Could you check a few things on this model? Use its own coordinates, in mm. A direction names the side the tool comes from. Round coordinates to 2 decimals unless told otherwise and drop trailing zeros. Loops run counter-clockwise (first coordinate to the right, second up) from the corner with the lowest first, then second, coordinate; pieces in that order, holes last. Notation, with made-up numbers: (84.25, -1.75) -> (138.25, -1.75) arc R13 ccw to (138.25, 9.25) -> close; hole circle Ø5 at (-34.5, -33.5). An arc over 180 degrees is marked (long way). One line per item, written item: value.
```python
from build123d import *

# Parameters (mm, degrees)
BASE_PLATE_DEPTH              = 75
BOSS_60_SKETCH_R              = 30
BOSS_60_DEPTH                 = 25
HUB_40_SKETCH_R               = 20
HUB_40_DEPTH                  = 20
BOLT_CIRCLE_8X_4_SKETCH_R     = 2
BOLT_CIRCLE_HOLES_8X_4_DEPTH  = 20
BORE_24_SKETCH_R              = 12
BORE_24_DEPTH                 = 210.652092763
MOUNTING_HOLES_4X_14_SKETCH_R = 7
MOUNTING_HOLES_4X_14_DEPTH    = 20
REINFORCING_RIB_A_REACH       = 201.337
RIB_A_SKETCH_WALL_W           = 489.696521402
RIB_A_SKETCH_WALL_H           = 10
REINFORCING_RIB_B_REACH       = 201.337
RIB_B_SKETCH_WALL_W           = 489.696521402
RIB_B_SKETCH_WALL_H           = 10


with BuildPart() as part:
    # Base Plate Profile → Base Plate (new body)
    with BuildSketch(Plane.XY):
        Polygon((0, 0), (50, 0), (50, 20), (130, 20), (130, 0), (180, 0), (180, 12), (142, 12), (142, 32), (38, 32), (38, 12), (0, 12), align=None)
    extrude(amount=-BASE_PLATE_DEPTH)

    # Boss Ø60 Sketch → Boss Ø60 (add)
    with BuildSketch(Plane(origin=(0, 32, 0), x_dir=(1, 0, 0), z_dir=(0, 1, 0))):
        with Locations(Location((90, 37.5, 0), (0, 0, 270))):
            Circle(BOSS_60_SKETCH_R)
    extrude(amount=BOSS_60_DEPTH)

    # Hub Ø40 Sketch → Hub Ø40 (add)
    with BuildSketch(Plane(origin=(0, 57, 0), x_dir=(1, 0, 0), z_dir=(0, 1, 0))):
        with Locations(Location((90, 37.5, 0), (0, 0, 270))):
            Circle(HUB_40_SKETCH_R)
    extrude(amount=HUB_40_DEPTH)

    # Bolt Circle 8xØ4 Sketch → Bolt Circle Holes 8xØ4 (cut)
    with BuildSketch(Plane(origin=(0, 77, 0), x_dir=(1, 0, 0), z_dir=(0, 1, 0))):
        with Locations(Location((90, 53.5, 0), (0, 0, 270))):
            Circle(BOLT_CIRCLE_8X_4_SKETCH_R)
        with Locations(Location((101.313708499, 48.813708499, 0), (0, 0, 270))):
            Circle(BOLT_CIRCLE_8X_4_SKETCH_R)
        with Locations(Location((106, 37.5, 0), (0, 0, 270))):
            Circle(BOLT_CIRCLE_8X_4_SKETCH_R)
        with Locations(Location((101.313708499, 26.186291501, 0), (0, 0, 270))):
            Circle(BOLT_CIRCLE_8X_4_SKETCH_R)
        with Locations(Location((90, 21.5, 0), (0, 0, 270))):
            Circle(BOLT_CIRCLE_8X_4_SKETCH_R)
        with Locations(Location((78.686291501, 26.186291501, 0), (0, 0, 270))):
            Circle(BOLT_CIRCLE_8X_4_SKETCH_R)
        with Locations(Location((74, 37.5, 0), (0, 0, 270))):
            Circle(BOLT_CIRCLE_8X_4_SKETCH_R)
        with Locations(Location((78.686291501, 48.813708499, 0), (0, 0, 270))):
            Circle(BOLT_CIRCLE_8X_4_SKETCH_R)
    extrude(amount=-BOLT_CIRCLE_HOLES_8X_4_DEPTH, mode=Mode.SUBTRACT)

    # Bore Ø24 Sketch → Bore Ø24 (cut, through all)
    with BuildSketch(Plane(origin=(0, 77, 0), x_dir=(1, 0, 0), z_dir=(0, 1, 0))):
        with Locations(Location((90, 37.5, 0), (0, 0, 270))):
            Circle(BORE_24_SKETCH_R)
    extrude(amount=-BORE_24_DEPTH, mode=Mode.SUBTRACT)

    # Mounting Holes 4xØ14 Sketch → Mounting Holes 4xØ14 (cut)
    with BuildSketch(Plane(origin=(0, 12, 0), x_dir=(1, 0, 0), z_dir=(0, 1, 0))):
        with Locations(Location((165, 60, 0), (0, 0, 270))):
            Circle(MOUNTING_HOLES_4X_14_SKETCH_R)
        with Locations(Location((165, 15, 0), (0, 0, 270))):
            Circle(MOUNTING_HOLES_4X_14_SKETCH_R)
        with Locations(Location((15, 60, 0), (0, 0, 270))):
            Circle(MOUNTING_HOLES_4X_14_SKETCH_R)
        with Locations(Location((15, 15, 0), (0, 0, 270))):
            Circle(MOUNTING_HOLES_4X_14_SKETCH_R)
    extrude(amount=-MOUNTING_HOLES_4X_14_DEPTH, mode=Mode.SUBTRACT)

    # Rib A Sketch wall → Reinforcing Rib A (add, up to next)
    with BuildSketch(Plane(origin=(145, 39.5, -37.5), x_dir=(0.786318338822, -0.617821551932, 0), z_dir=(0.617821551932, 0.786318338822, 0)), mode=Mode.PRIVATE) as reinforcing_rib_a_sk1:
        Rectangle(RIB_A_SKETCH_WALL_W, RIB_A_SKETCH_WALL_H)
    reinforcing_rib_a_tool1 = extrude(reinforcing_rib_a_sk1.sketch, amount=-REINFORCING_RIB_A_REACH, mode=Mode.PRIVATE) - part.part
    add(reinforcing_rib_a_tool1.solids().sort_by_distance((145, 39.5, -37.5))[0])

    # Rib B Sketch wall → Reinforcing Rib B (add, up to next)
    with BuildSketch(Plane(origin=(35, 39.5, -37.5), x_dir=(-0.786318338822, -0.617821551932, 0), z_dir=(0.617821551932, -0.786318338822, 0)), mode=Mode.PRIVATE) as reinforcing_rib_b_sk1:
        Rectangle(RIB_B_SKETCH_WALL_W, RIB_B_SKETCH_WALL_H)
    reinforcing_rib_b_tool1 = extrude(reinforcing_rib_b_sk1.sketch, amount=REINFORCING_RIB_B_REACH, mode=Mode.PRIVATE) - part.part
    add(reinforcing_rib_b_tool1.solids().sort_by_distance((35, 39.5, -37.5))[0])


solid = part.part
```
(1) Imagine slicing it at B-B on z = -37.5. Write out the boundary of the cut face in (x, y).
Results below:
outline: (0, 0) -> (50, 0) -> (50, 20) -> (78, 20) -> (78, 77) -> (76, 77) -> (76, 57) -> (72, 57) -> (72, 77) -> (70, 77) -> (70, 67) -> (0, 12) -> close; (102, 20) -> (130, 20) -> (130, 0) -> (180, 0) -> (180, 12) -> (110, 67) -> (110, 77) -> (108, 77) -> (108, 57) -> (104, 57) -> (104, 77) -> (102, 77) -> close
(2) We'd pull the mould along Z, two halves only. Please class faces 6 (the face through (89, 23, 0)), 7 (the face through (130, 10, -37)), 8 (the face through (10.741, 6.084, -20.555)): +Z half, -Z half, draft (parallel to the pull), parting line (faces both ways), or undercut.
Results below:
face 6: +Z half
face 7: draft
face 8: undercut
(3) Imagine slicing it at C-C on y = 45. Write out the boundary of the cut face in (x, z).
Results below:
outline: (42, -42.5) -> (60.42, -42.5) arc R30 ccw to (119.58, -42.5) -> (138, -42.5) -> (138, -32.5) -> (119.58, -32.5) arc R30 ccw to (60.42, -32.5) -> (42, -32.5) -> close; hole circle Ø24 at (90, -37.5)
(4) Imagine slicing it at D-D on z = -15. Write out the boundary of the cut face in (x, y), then the cut area to 3 significant figures.
Results below:
outline: (0, 0) -> (8, 0) -> (8, 12) -> (0, 12) -> close; (22, 0) -> (50, 0) -> (50, 20) -> (130, 20) -> (130, 0) -> (158, 0) -> (158, 12) -> (142, 12) -> (142, 32) -> (109.84, 32) -> (109.84, 57) -> (70.16, 57) -> (70.16, 32) -> (38, 32) -> (38, 12) -> (22, 12) -> close; (172, 0) -> (180, 0) -> (180, 12) -> (172, 12) -> close
area: 3,300 mm²
(5) On a 3-axis mill with a long thin cutter (end or side, diameter ignored), from which of +Z, -Z, +X, -X, +Y, -Y can I reach the whole of each face in a straight line? I mean faces 1 (the face through (91, 32, -5)), 2 (the face through (90.589, 44.325, -67.494)), 3 (the face through (50, 10, -37)), 4 (the face through (76.734, 67.14, -26.62)), 5 (the face through (38, 22, -16)). Say none if no direction works.
Results below:
face 1: +Z, +Y
face 2: -Z, +Y
face 3: +Z, -Z, -Y
face 4: +Y
face 5: +Z, -X, +Y
(6) Imagine slicing it at A-A on x = 90. Write out the boundary of the cut face in (y, z).
Results below:
outline: (20, -75) -> (32, -75) -> (32, -67.5) -> (57, -67.5) -> (57, -57.5) -> (77, -57.5) -> (77, -55.5) -> (57, -55.5) -> (57, -51.5) -> (77, -51.5) -> (77, -49.5) -> (20, -49.5) -> close; (20, -25.5) -> (77, -25.5) -> (77, -23.5) -> (57, -23.5) -> (57, -19.5) -> (77, -19.5) -> (77, -17.5) -> (57, -17.5) -> (57, -7.5) -> (32, -7.5) -> (32, 0) -> (20, 0) -> close
(7) For pin 1 Ø1 at (y, z) = (54, -33.5) entering from +X; pin 2 Ø2.5 at (x, z) = (78.69, -48.81) entering from -Y; pin 3 Ø1 at (y, z) = (66, -46) entering from +X; pin 4 Ø3 at (x, z) = (105.5, -38) entering from +Y, each with a flat end and sliding along its axis, tell me the tip position at first contact or that it passes through.
Results below:
pin 1: stops at x = 127.18
pin 2: stops at y = 20
pin 3: stops at x = 108.33
pin 4: stops at y = 77
(8) Please list where these lines run through material, in increasing order: L1, parallel to X at y = 63, z = -37.5; L2, parallel to Y at x = 132, z = -64; L3, parallel to Y at x = 68, z = -57.
Results below:
L1: x = 64.91 to 72, 76 to 78, 102 to 104, 108 to 115.09
L2: y = 0 to 32
L3: y = 20 to 57
